Print and shaded views of the part. All mm, measured from the part's lowest x, y and z. A direction names the side the tool comes from. Round coordinates to 2 decimals unless told otherwise and drop trailing zeros. Write each loop counter-clockwise with the first axis right and the second up, starting at its lowest first coordinate (ties: lowest second). Pieces come first, ordered by that corner, then holes. Notation, with made-up numbers: M 25.5,26.25 L 32.5,26.25 A28 ccw 32.5,60.25 Z; hole C 12.25,-19 d11. An arc over 180 degrees is marked long. Write item = value, one per line.
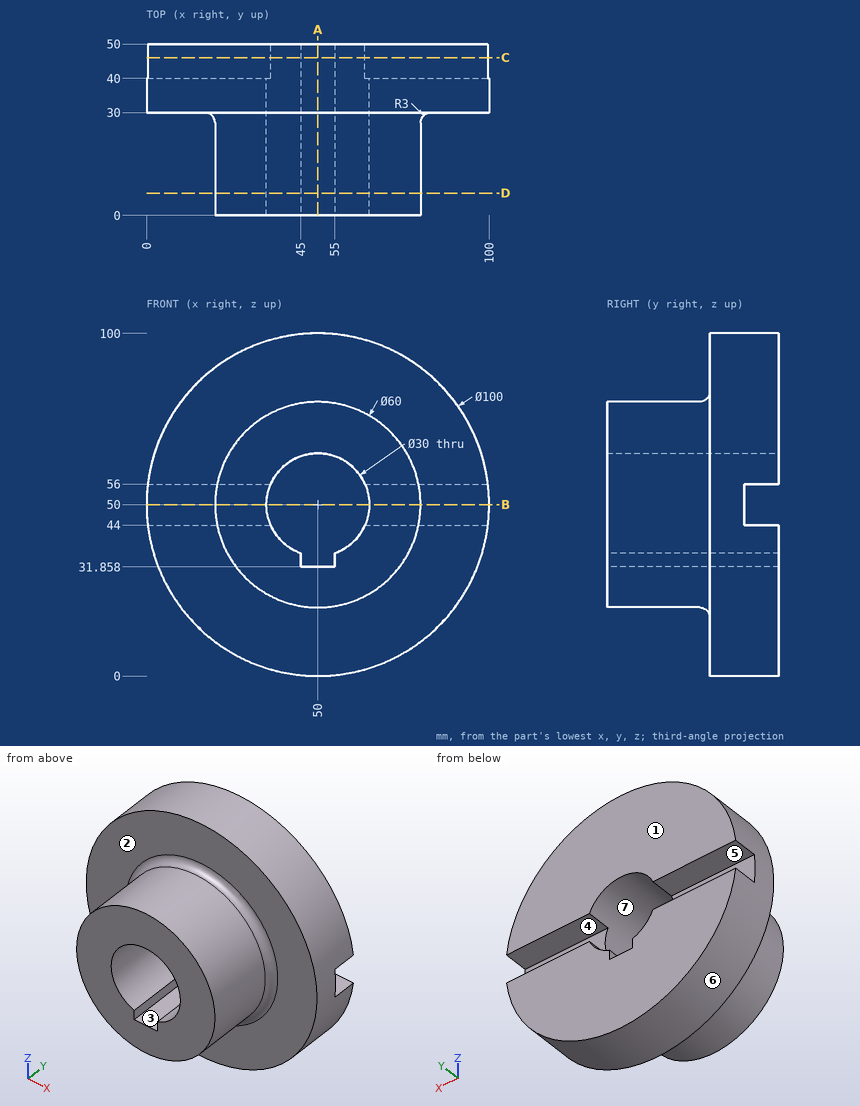
1. Band-saw the part on D-D (y = 6.5). List the corners of the cut face in (x, z), plus the area to 3 significant figures.
Responses:
outline = C 50,50 d60; hole M 45,31.86 L 55,31.86 L 55,35.86 A15 ccw long 45,35.86 Z
area = 2,090 mm²
2. Probe probe 1 along Z at (x, y) = (50, 21.5); probe 2 along X at (y, z) = (34, 50); probe 3 along X at (y, z) = (11.5, 50). List the from-to ranges inside material, lowest first.
Responses:
probe_1 = 20 to 31.86, 65 to 80
probe_2 = 0 to 35, 65 to 100
probe_3 = 20 to 35, 65 to 80
3. Flat gauge pins, fed straight in: pin 1 (1.2 mm diameter, centred on y = 25, z = 34, fed in from -X); pin 2 (11 mm diameter, centred on x = 12, y = 47, fed in from +Z); pin 3 (5 mm diameter, centred on x = 24, z = 52, fed in from +Y); pin 4 (5 mm diameter, centred on x = 52.5, y = 30.5, fed in from +Z). Where does each tip first touch, or does it go through?
Responses:
pin_1 = 24.25
pin_2 = 88
pin_3 = 40
pin_4 = 100
4. Band-saw the part on A-A (x = 50). List the corners of the cut face in (y, z), plus the area to 3 significant figures.
Responses:
outline = M 0,20 L 27,20 A3 cw 30,17 L 30,0 L 50,0 L 50,31.86 L 0,31.86 Z; M 0,65 L 50,65 L 50,100 L 30,100 L 30,83 A3 cw 27,80 L 0,80 Z
area = 2,150 mm²
5. Tool access for the marked faces 1, 2, 3 and 4: list every direction of +Z, -Z, +X, -X, +Y, -Y with a clear straight run to the whole face (end or side of a thin tool).
Responses:
face_1 = +Z, -Z, +X, -X, +Y
face_2 = -Y
face_3 = +Y, -Y
face_4 = +X, -X, +Y
6. Band-saw the part on C-C (y = 46). List the corners of the cut face in (x, z).
Responses:
outline = M 0.36,44 A50 ccw 99.64,44 L 63.75,44 A15 cw 55,35.86 L 55,31.86 L 45,31.86 L 45,35.86 A15 cw 36.25,44 Z; M 0.36,56 L 36.25,56 A15 cw 63.75,56 L 99.64,56 A50 ccw Z
7. Mould opens along X. For the marked faces 5, 6 and 7 say: pulls with the +X half, pulls with the -X half, needs draft (parallel to the pull), parting line crosses it, or undercut.
Responses:
face_5 = needs draft
face_6 = parting line crosses it
face_7 = undercut
8. Band-saw the part on B-B (z = 50). List the corners of the cut face in (x, y), plus the area to 3 significant figures.
Responses:
outline = M 0,30 L 17,30 A3 cw 20,27 L 20,0 L 35,0 L 35,40 L 0,40 Z; M 65,0 L 80,0 L 80,27 A3 cw 83,30 L 100,30 L 100,40 L 65,40 Z
area = 1,600 mm²
